Here's how the part is built. I have some questions about the finished solid (model axes, mm). Round coordinates to 2 decimals unless told otherwise and drop trailing zeros. Loops run counter-clockwise (first coordinate to the right, second up) from the corner with the lowest first, then second, coordinate; pieces in that order, holes last. Notation, with made-up numbers: (-5.5, 69) - (17.5, 69) arc R29 ccw to (17.5, 94) - close; hole circle Ø6 at (71.5, 23.25). An arc over 180 degrees is marked (long way). Answer as a JSON object with one key per item and string values. Group by question number.
1) I want a section at C-C, the plane z = 20. Please give me the cut outline in (x, y).
2) If I drill on line 1 along Y through (x, z) = (150, 14.75); line 2 along X through (y, z) = (164, 19.5); line 3 along Y through (x, z) = (171.5, 3.75), over which ranges is the centre line in solid material (lowest first)? Write a range as [from, to].
3) I want a section at A-A, the plane x = 150. Please give me the cut outline in (y, z).
4) If we mould it in two halves opening along X, with no side actions, what happens to faces 1 (the face through (0, 277, 12)), 2 (the face through (262.56, 280.51, 12.68)), 3 (the face through (297, 303, 12))? For each: pulls with the +X half, pulls with the -X half, needs draft (parallel to the pull), parting line crosses it, or undercut.
5) I want a section at D-D, the plane y = 440. Please give me the cut outline in (x, z).
6) Will these pins go through, and if not, where does the flat tip stop? P1, Ø12, axis at x = 129, y = 291.5, coming from the -Z side; P2, Ø10, axis at y = 52.5, z = 17, coming from the -X side; P3, Ø10, axis at x = 381.5, z = 11.5, coming from the +Y side; P4, Ø1, axis at y = 442.5, z = 11.5, coming from the +X side.
from build123d import *

# Parameters (mm, degrees)
BOSS_EXTRUDE1_DEPTH = 25
SKETCH2_R           = 25
CUT_EXTRUDE1_DEPTH  = 25
CHAMFER1_SIZE       = 60
SKETCH3_R           = 16
CUT_EXTRUDE2_DEPTH  = 708.548584904


with BuildPart() as part:
    # Sketch1 → Boss-Extrude1 (new body)
    with BuildSketch(Plane.XY):
        Polygon((0, 0), (0, 500), (100, 500), (500, 100), (500, 0), align=None)
    extrude(amount=BOSS_EXTRUDE1_DEPTH)

    # Sketch2 → Cut-Extrude1 (cut)
    with BuildSketch(Plane.XY.offset(25)):
        with Locations((150, 150)):
            Circle(SKETCH2_R)
    extrude(amount=-CUT_EXTRUDE1_DEPTH, mode=Mode.SUBTRACT)

    # Chamfer1
    chamfer1_edges = [part.edges().sort_by_distance(p)[0] for p in [
        (0, 0, 12.5),
    ]]
    chamfer(chamfer1_edges, length=CHAMFER1_SIZE)

    # Sketch3 → Cut-Extrude2 (cut, through all)
    with BuildSketch(Plane.XY.offset(25)):
        with Locations((264.644660941, 264.644660941)):
            Circle(SKETCH3_R)
    extrude(amount=-CUT_EXTRUDE2_DEPTH, mode=Mode.SUBTRACT)


solid = part.part
Outcome:
{
 "1": {"outline": "(0, 60) - (60, 0) - (500, 0) - (500, 100) - (100, 500) - (0, 500) - close; hole circle Ø50 at (150, 150); hole circle Ø32 at (264.64, 264.64)"},
 "2": {"line 1": "[0, 125], [175, 450]", "line 2": "[0, 129.29], [170.71, 436]", "line 3": "[0, 137.24], [162.76, 428.5]"},
 "3": {"outline": "(0, 0) - (125, 0) - (125, 25) - (0, 25) - close; (175, 0) - (450, 0) - (450, 25) - (175, 25) - close"},
 "4": {"face 1": "pulls with the -X half", "face 2": "undercut", "face 3": "pulls with the +X half"},
 "5": {"outline": "(0, 0) - (160, 0) - (160, 25) - (0, 25) - close"},
 "6": {"P1": "z = 0", "P2": "x = 2.5", "P3": "y = 223.5", "P4": "x = 158"}
}
